Here's how the part is built. I have some questions about the finished solid (model axes, mm). Face numbers are marked on the shaded views. A direction names the side the tool comes from. Give positions to 0.01 mm unless a question says otherwise; leave off trailing zeros. Order: outer loops, then holes, each group sorted by start corner. A loop starts at its lowest first (then second) coordinate and runs counter-clockwise, first axis right, second up. Notation, with made-up numbers: M 21,3 L 52,3 A28 cw 52,40 Z; hole C -5.75,24 d9. An arc over 180 degrees is marked long. One line per item, written item: value. Start each with the question number.
from build123d import *

# Parameters (mm, degrees)
SKETCH1_R           = 6
BOSS_EXTRUDE1_DEPTH = 28.65
SKETCH2_R           = 10
BOSS_EXTRUDE2_DEPTH = 12.1
SKETCH3_R           = 10.5
BOSS_EXTRUDE3_DEPTH = 1
SKETCH4_R           = 6
BOSS_EXTRUDE4_DEPTH = 48.6
CUT_EXTRUDE1_DEPTH  = 0.9


with BuildPart() as part:
    # Sketch1 → Boss-Extrude1 (new body)
    with BuildSketch(Plane.XY):
        Circle(SKETCH1_R)
    extrude(amount=BOSS_EXTRUDE1_DEPTH)

    # Sketch2 → Boss-Extrude2 (add)
    with BuildSketch(Plane.XY.offset(28.65)):
        Circle(SKETCH2_R)
    extrude(amount=BOSS_EXTRUDE2_DEPTH)

    # Sketch3 → Boss-Extrude3 (add)
    with BuildSketch(Plane.XY.offset(40.75)):
        Circle(SKETCH3_R)
    extrude(amount=BOSS_EXTRUDE3_DEPTH)

    # Sketch4 → Boss-Extrude4 (add)
    with BuildSketch(Plane.XY.offset(41.75)):
        Circle(SKETCH4_R)
    extrude(amount=BOSS_EXTRUDE4_DEPTH)

    # Sketch6 → Cut-Extrude1 (cut, symmetric)
    with BuildSketch(Plane(origin=(0, 10, 0), x_dir=(1, 0, 0), z_dir=(0, 1, 0))):
        with BuildLine():
            Line((1.5, -32.25), (1.5, -37.25))
            ThreePointArc((1.5, -37.25), (0, -38.75), (-1.5, -37.25))
            Line((-1.5, -37.25), (-1.5, -32.25))
            ThreePointArc((-1.5, -32.25), (0, -30.75), (1.5, -32.25))
        make_face()
    extrude(amount=CUT_EXTRUDE1_DEPTH, both=True, mode=Mode.SUBTRACT)


solid = part.part
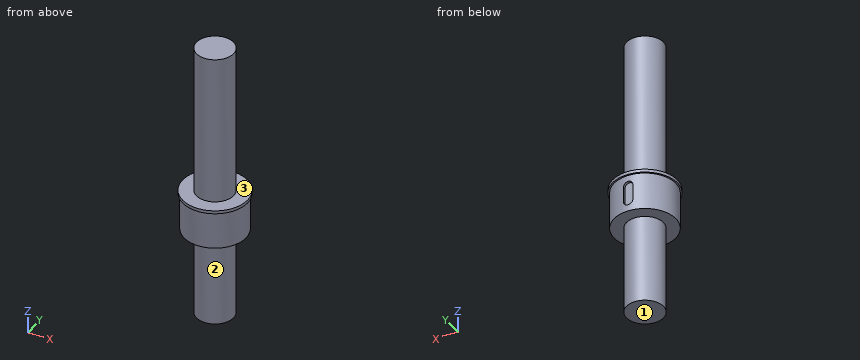
Item 1: Please list where these lines run through material, in increasing order: probe 1 along Z at (x, y) = (7.25, 6); probe 2 along Y at (x, z) = (-0.25, 23.5); probe 3 along X at (y, z) = (3.5, 6). Write a range as [from, to].
Item 2: I want a section at C-C on z = 19.5. Write out the boundary of the cut face in (x, y), plus the area to 3 significant figures.
Item 3: Will these pins go through, and if not, where does the flat tip stop? P1, Ø12, axis at x = 0.5, y = 0, coming from the -Z side; P2, Ø12, axis at x = 5.5, z = 14.5, coming from the +Y side; P3, Ø3, axis at x = 4.5, z = 46.5, coming from the +Y side; P4, Ø3.5, axis at x = 0, z = 35, coming from the +Y side.
Item 4: I want a section at D-D on x = 8.75. Write out the boundary of the cut face in (y, z).
Item 5: I want a section at A-A on y = 0. Write out the boundary of the cut face in (x, z), plus the area to 3 significant figures.
Item 6: For the marked faces 1, 2 and 3, which set-ups out of +Z, -Z, +X, -X, +Y, -Y let a thin tool reach every point of the face, with its end or its side?
Item 7: I want a section at B-B on x = -3. Write out the boundary of the cut face in (y, z), plus the area to 3 significant figures.
Answer below:
1. probe 1: z = [28.65, 41.75]
1. probe 2: y = [-5.99, 5.99]
1. probe 3: x = [-4.87, 4.87]
2. outline: C 0,0 d12
2. area: 113 mm²
3. P1: stops at z = 0
3. P2: stops at y = 6
3. P3: stops at y = 5.2
3. P4: stops at y = 9.89
4. outline: M -5.8,40.75 L -4.84,40.75 L -4.84,28.65 L 4.84,28.65 L 4.84,40.75 L 5.8,40.75 L 5.8,41.75 L -5.8,41.75 Z
5. outline: M -10.5,40.75 L -10,40.75 L -10,28.65 L -6,28.65 L -6,0 L 6,0 L 6,28.65 L 10,28.65 L 10,40.75 L 10.5,40.75 L 10.5,41.75 L 6,41.75 L 6,90.35 L -6,90.35 L -6,41.75 L -10.5,41.75 Z
5. area: 1,190 mm²
6. face 1: -Z, +X, -X, +Y, -Y
6. face 2: -Z
6. face 3: +Z
7. outline: M -10.06,40.75 L -9.54,40.75 L -9.54,28.65 L -5.2,28.65 L -5.2,0 L 5.2,0 L 5.2,28.65 L 9.54,28.65 L 9.54,40.75 L 10.06,40.75 L 10.06,41.75 L 5.2,41.75 L 5.2,90.35 L -5.2,90.35 L -5.2,41.75 L -10.06,41.75 Z
7. area: 1,050 mm²
